Geometry: see drawing. Coordinates: mm, zero at the bounding-box minimum. A direction names the side the tool comes from. Round coordinates to 2 decimals unless told otherwise and drop trailing zeros. Write each loop counter-clockwise with the first axis right and the second up, starting at its lowest first coordinate (ties: lowest second). Pieces come first, ordered by that corner, then holes. Notation, with made-up numbers: M 57.5,-4.5 L 113.5,-4.5 A5 cw 113.5,1.5 Z; hole C 28,-36 d3. An arc over 180 degrees is marked long. Use one line per item in the form item = value. Start each with the question number.
Item 1: Section query D-D (x = 43.5). Return loops of the section in (y, z), and give its area (3 significant figures).
Item 2: Pin query (flat end, axial travel): pin 1 Ø4 at (x, y) = (18, 48.5) entering from +Z; pin 2 Ø3 at (x, y) = (14.5, 11.5) entering from +Z; pin 3 Ø2 at (x, y) = (23, 47) entering from -Z; pin 4 Ø6 at (y, z) = (69.5, 50.5) entering from -X. Return the tip coordinate at first contact, or that it passes through.
Item 3: Section query C-C (x = 8.5). Return loops of the section in (y, z).
Item 4: Pull-direction query (Y, two-part tool) for the marked faces 4, 5 and 6; classes: pulls with the +Y half, pulls with the -Y half, needs draft (parallel to the pull), parting line crosses it, or undercut.
Item 5: Section query A-A (y = 40). Return loops of the section in (x, z) (1 decimal).
Item 6: Reachability of the marked faces 1, 2 and 3 from +Z, -Z, +X, -X, +Y, -Y: full face, straight path, thin tool, end or side. Return the list, or none.
Item 7: Ray query, probe 1 along Y at (x, z) = (20, 40); probe 2 along X at (y, z) = (7, 39) (1 decimal); probe 3 along X at (y, z) = (60.5, 65). Return the intervals inside material, ascending.
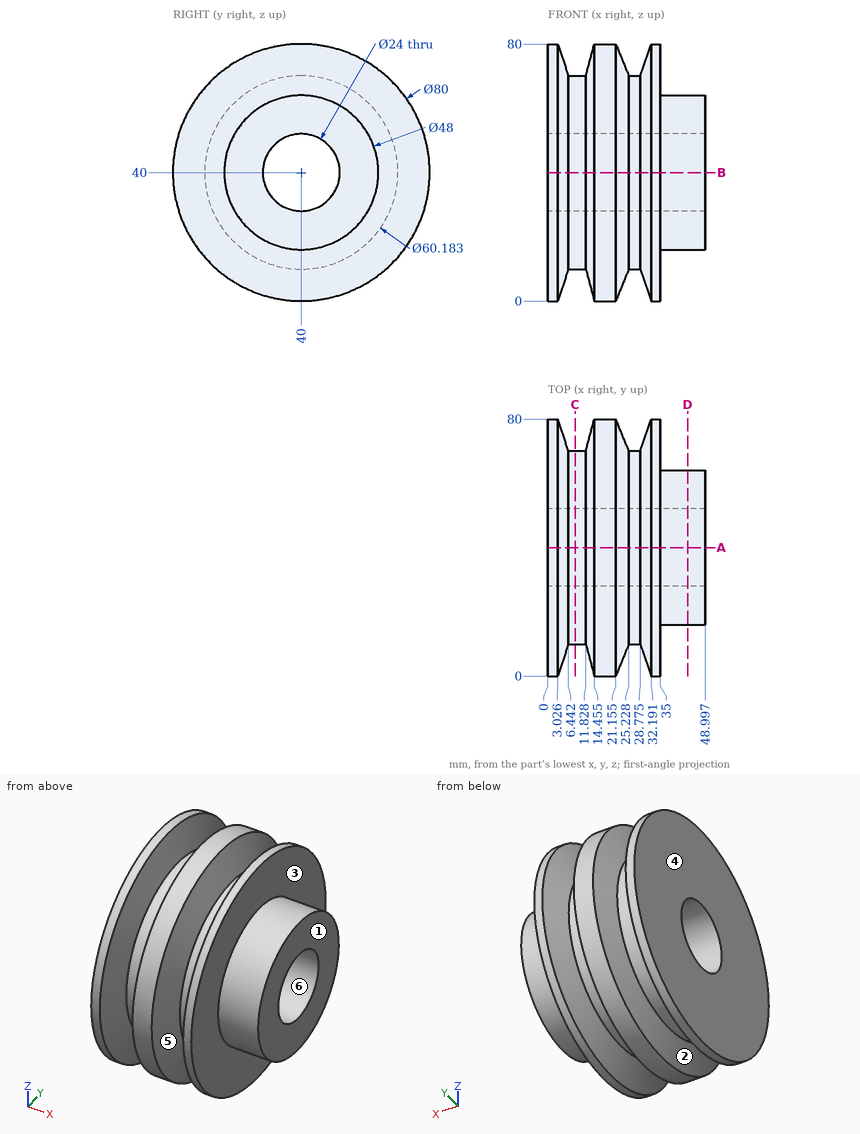
Working result:
q1.outline = C 40,40 d48; hole C 40,40 d24
q1.area = 1,360 mm²
q2.pin_1 = 79.47
q2.pin_2 = 69.51
q2.pin_3 = 2.7
q2.pin_4 = 0
q3.outline = C 40,40 d60.18; hole C 40,40 d24
q4.face_4 = needs draft
q4.face_5 = parting line crosses it
q4.face_6 = undercut
q5.outline = M 0,0 L 3,0 L 6.4,9.9 L 11.8,9.9 L 14.5,0 L 21.2,0 L 25.2,9.9 L 28.8,9.9 L 32.2,0 L 35,0 L 35,16 L 49,16 L 49,28 L 0,28 Z; M 0,52 L 49,52 L 49,64 L 35,64 L 35,80 L 32.2,80 L 28.8,70.1 L 25.2,70.1 L 21.2,80 L 14.5,80 L 11.8,70.1 L 6.4,70.1 L 3,80 L 0,80 Z
q6.face_1 = +Z, -Z, +X, +Y, -Y
q6.face_2 = none
q6.face_3 = +X
q7.probe_1 = 0 to 28, 52 to 80
q7.probe_2 = 0 to 5.4, 12.6 to 24, 29.8 to 35
q7.probe_3 = 0 to 5.67, 12.42 to 24.31, 29.55 to 35
